The model under review builds one solid part; all positions refer to its coordinate system, in mm. Face numbers are marked on the shaded views. A direction names the side the tool comes from. Coordinates: 2 decimals unless noted, no trailing zeros. Loops run counter-clockwise (first coordinate to the right, second up) from the corner with the lowest first, then second, coordinate; pieces in that order, holes last. Notation, with made-up numbers: (68.25, 71.25) - (107.25, 71.25) arc R35 ccw to (107.25, 106.25) - close; hole circle Ø4 at (70, 38.5). An arc over 180 degrees is marked (long way). Use a Markdown table: item, result. Add a question column.
1) Clearance check with flat-ended pins moving along their axes: pin 1 (3 mm diameter, centred on x = -5.5, z = 10, fed in from +Y); pin 2 (5 mm diameter, centred on y = 3.5, z = 29.5, fed in from -X); pin 3 (8 mm diameter, centred on x = 5, y = 38.5, fed in from +Z); pin 4 (9 mm diameter, centred on y = 4, z = 30, fed in from +X). State where each tip first meets the part, or that it passes through.
2) Add section D-D, the plane y = 30.5. Give the boundary of the cut face in (x, z), and give its area (3 significant figures).
3) Add section C-C, the plane z = -30. Give the boundary of the cut face in (x, y), and give its area (3 significant figures).
4) Add section A-A, the plane z = 30. Give the boundary of the cut face in (x, y), and give its area (3 significant figures).
5) To check wall thickness, follow L1, parallel to Y at x = 0, z = -32.5; L2, parallel to Y at x = -4.75, z = 3; L3, parallel to Z at x = -3.5, y = 3. State the ranges of each line that lie inside material, in increasing order. Write a range as [from, to].
6) For the marked faces 4 and 5, list the 3-axis set-ups (+Z, -Z, +X, -X, +Y, -Y) from which the entire face can be reached by the end or side of a thin tool; tool diameter is ignored.
7) Add section B-B, the plane x = -5. Give the boundary of the cut face in (y, z), and give its area (3 significant figures).
8) The part is to be moulded in two halves that separate along Z. For the marked faces 1, 2 and 3, say which applies: pulls with the +Z half, pulls with the -Z half, needs draft (parallel to the pull), parting line crosses it, or undercut.
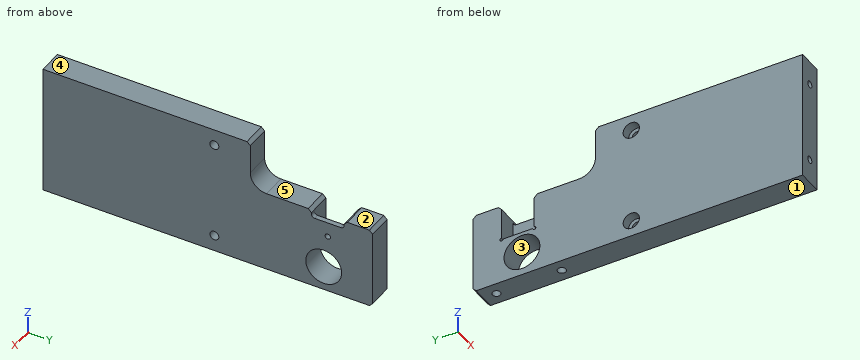
```python
from build123d import *

# Parameters (mm, degrees)
EXTRUDE_1_DEPTH                = 7.5
SKETCH_2_R                     = 11
CUT_EXTRUDE_1_DEPTH            = 110.66312051
HOLE_WIZARD_M5_1_D             = 4.2
HOLE_WIZARD_M5_1_DEPTH         = 12.4
HOLE_WIZARD_M5_1_TIP           = 1.2618073
HOLE_WIZARD_M5_1_2_D           = 5.5
HOLE_WIZARD_M5_1_2_CBORE_D     = 10
HOLE_WIZARD_M5_1_2_CBORE_DEPTH = 5.7
HOLE_WIZARD_M6_1_D             = 5
HOLE_WIZARD_M6_1_DEPTH         = 15
HOLE_WIZARD_M6_1_TIP           = 1.502151548
CHAMFER_1_SIZE                 = 2
SKETCH_12_R                    = 2.5
CUT_EXTRUDE_2_DEPTH            = 110.66312051
HOLE_WIZARD_M4_1_D             = 3.3
SKETCH_15_W                    = 22
SKETCH_15_H                    = 20
CUT_EXTRUDE_3_DEPTH            = 12
SKETCH_16_W                    = 5
SKETCH_16_H                    = 20
CUT_EXTRUDE_4_DEPTH            = 110.293183685
SKETCH_17_R                    = 1
CUT_EXTRUDE_5_DEPTH            = 12
CHAMFER_2_SIZE                 = 2
FILLET_2_R                     = 2


with BuildPart() as part:
    # 草图1 → 凸台-拉伸1 (new, symmetric)
    with BuildSketch(Plane(origin=(0, 0, 0), x_dir=(0, 0, -1), z_dir=(1, 0, 0))):
        with BuildLine():
            Line((-10, 101), (-10, 36))
            ThreePointArc((-10, 36), (-12.928932188, 28.928932188), (-20, 26))
            Line((-20, 26), (-40, 26))
            Line((-40, 26), (-40, -101))
            Line((-40, -101), (40, -101))
            Line((40, -101), (40, 101))
            Line((40, 101), (-10, 101))
        make_face()
    extrude(amount=EXTRUDE_1_DEPTH, both=True)

    # 草图2 → 切除-拉伸1 (cut, through all)
    with BuildSketch(Plane.ZY.offset(7.5)):
        with Locations((-25, 71)):
            Circle(SKETCH_2_R)
    extrude(amount=-CUT_EXTRUDE_1_DEPTH, mode=Mode.SUBTRACT)

    # Hole Wizard M5 _1
    with Locations(Plane(origin=(0, -101, 0), x_dir=(-1, 0, 0), z_dir=(0, -1, 0))):
        with Locations((0, 25), (0, -25)):
            Hole(HOLE_WIZARD_M5_1_D / 2, depth=HOLE_WIZARD_M5_1_DEPTH)
            with Locations((0, 0, -(HOLE_WIZARD_M5_1_DEPTH + HOLE_WIZARD_M5_1_TIP / 2))):  # 118° drill point
                Cone(0, HOLE_WIZARD_M5_1_D / 2, HOLE_WIZARD_M5_1_TIP, mode=Mode.SUBTRACT)

    # Hole Wizard M5 _1 2 (through all)
    with Locations(Plane.ZY.offset(7.5)):
        with Locations((-30, 4), (30, 4)):
            CounterBoreHole(HOLE_WIZARD_M5_1_2_D / 2, HOLE_WIZARD_M5_1_2_CBORE_D / 2, HOLE_WIZARD_M5_1_2_CBORE_DEPTH)

    # M6 螺纹孔1
    with Locations(Plane(origin=(0, 0, -40), x_dir=(-1, 0, 0), z_dir=(0, 0, -1))):
        with Locations((0, 51), (0, 91)):
            Hole(HOLE_WIZARD_M6_1_D / 2, depth=HOLE_WIZARD_M6_1_DEPTH)
            with Locations((0, 0, -(HOLE_WIZARD_M6_1_DEPTH + HOLE_WIZARD_M6_1_TIP / 2))):  # 118° drill point
                Cone(0, HOLE_WIZARD_M6_1_D / 2, HOLE_WIZARD_M6_1_TIP, mode=Mode.SUBTRACT)

    # 倒角1
    chamfer_1_edges = [part.edges().sort_by_distance(p)[0] for p in [
        (0, 26, 40),
        (0, 101, 10),
        (0, 101, -40),
    ]]
    chamfer(chamfer_1_edges, length=CHAMFER_1_SIZE)

    # 草图12 → 切除-拉伸2 (cut, through all)
    with BuildSketch(Plane(origin=(7.5, 0, 0), x_dir=(0, 0, -1), z_dir=(1, 0, 0))):
        with Locations((-11, 73.5)):
            Circle(SKETCH_12_R)
    extrude(amount=-CUT_EXTRUDE_2_DEPTH, mode=Mode.SUBTRACT)

    # M4 螺纹孔1 (through all)
    with Locations(Plane.ZY.offset(7.5)):
        with Locations((-4, 73.5)):
            Hole(HOLE_WIZARD_M4_1_D / 2)

    # 草图15 → 切除-拉伸3 (cut)
    with BuildSketch(Plane.ZY.offset(7.5)):
        with Locations((-1, 73.5)):
            Rectangle(SKETCH_15_W, SKETCH_15_H)
    extrude(amount=-CUT_EXTRUDE_3_DEPTH, mode=Mode.SUBTRACT)

    # 草图16 → 切除-拉伸4 (cut, through all)
    with BuildSketch(Plane.ZY.offset(-4.5)):
        with Locations((7.5, 73.5)):
            Rectangle(SKETCH_16_W, SKETCH_16_H)
    extrude(amount=-CUT_EXTRUDE_4_DEPTH, mode=Mode.SUBTRACT)

    # 草图17 → 切除-拉伸5 (cut)
    with BuildSketch(Plane.ZY.offset(7.5)):
        with Locations((-12, 83.5)):
            Circle(SKETCH_17_R)
        with Locations((-12, 63.5)):
            Circle(SKETCH_17_R)
    extrude(amount=-CUT_EXTRUDE_5_DEPTH, mode=Mode.SUBTRACT)

    # 倒角2
    chamfer_2_edges = [part.edges().sort_by_distance(p)[0] for p in [
        (0, 83.5, 10),
        (0, 63.5, 10),
    ]]
    chamfer(chamfer_2_edges, length=CHAMFER_2_SIZE)

    # 圆角2
    fillet_2_edges = [part.edges().sort_by_distance(p)[0] for p in [
        (6, 63.5, 5),
        (6, 83.5, 5),
    ]]
    fillet(fillet_2_edges, radius=FILLET_2_R)


solid = part.part
```
From the geometry:
| question | item | result |
|---|---|---|
| 1 | pin 1 | stops at y = 100.5 |
| 1 | pin 2 | stops at x = -1.8 |
| 1 | pin 3 | stops at z = 10.11 |
| 1 | pin 4 | stops at x = 7.5 |
| 2 | outline | (-7.5, -40) - (7.5, -40) - (7.5, 11.65) - (-7.5, 11.65) - close |
| 2 | area | 775 mm^2 |
| 3 | outline | (-7.5, -101) - (7.5, -101) - (7.5, 1.25) - (-1.8, 1.25) - (-1.8, -1) - (-7.5, -1) - close; (-7.5, 9) - (-1.8, 9) - (-1.8, 6.75) - (7.5, 6.75) - (7.5, 61.2) - (-7.5, 61.2) - close; (-7.5, 80.8) - (7.5, 80.8) - (7.5, 101) - (-7.5, 101) - close; hole circle Ø5 at (0, 51); hole circle Ø5 at (0, 91) |
| 3 | area | 2,590 mm^2 |
| 4 | outline | (-7.5, -101) - (7.5, -101) - (7.5, 1.25) - (-1.8, 1.25) - (-1.8, -1) - (-7.5, -1) - close; (-7.5, 9) - (-1.8, 9) - (-1.8, 6.75) - (7.5, 6.75) - (7.5, 26) - (-7.5, 26) - close |
| 4 | area | 1,800 mm^2 |
| 5 | L1 | y = [-101, 2.85], [5.15, 48.5], [53.5, 62.95], [79.05, 88.5], [93.5, 101] |
| 5 | L2 | y = [-101, 63.5], [83.5, 101] |
| 5 | L3 | z = [-40, -34.9], [-25.1, 25.1], [34.9, 40] |
| 6 | face 4 | +Z, +X, -X, +Y, -Y |
| 6 | face 5 | +Z, +X, -X, +Y |
| 7 | outline | (-101, -40) - (99, -40) - (101, -38) - (101, 8) - (99, 10) - (85.5, 10) - (83.5, 8) - (83.5, -11) arc R1 cw (long way) to (82.5, -12) - (64.5, -12) arc R1 cw (long way) to (63.5, -11) - (63.5, 8) - (61.5, 10) - (36, 10) arc R10 cw to (26, 20) - (26, 38) - (24, 40) - (-101, 40) - close; hole circle Ø10 at (4, -30); hole circle Ø10 at (4, 30); hole circle Ø22 at (71, -25) |
| 7 | area | 12,900 mm^2 |
| 8 | face 1 | pulls with the -Z half |
| 8 | face 2 | pulls with the +Z half |
| 8 | face 3 | undercut |
